Geometry: final body of the model. Coordinates: model frame, mm. Face numbers are marked on the shaded views. A direction names the side the tool comes from. Give positions to 0.01 mm unless a question says otherwise; leave off trailing zeros. Write each loop counter-clockwise with the first axis right and the second up, starting at its lowest first coordinate (ties: lowest second). Pieces come first, ordered by that corner, then holes. Notation, with made-up numbers: M 18.5,49.25 L 40.5,49.25 A34 cw 40.5,82.25 Z; hole C 52.25,89.5 d10. An arc over 180 degrees is marked long. Use one line per item in the form item = value. Start each with the question number.
Item 1: Section query A-A on y = 2.7. Return loops of the section in (x, z).
Item 2: Contact query for flat-ended pins moving along their axis: P1, Ø1.5, axis at y = 2.5, z = 1.5, coming from the -X side; P2, Ø1, axis at y = 4, z = 4, coming from the -X side. Output: stop coordinate, or through.
Item 3: Material intervals for line 1 along X through (y, z) = (2.75, 3); line 2 along Y through (x, z) = (4, 0.5); line 3 along X through (y, z) = (3.1, 2.1), sorted ascending. Write a range as from..to.
Item 4: Section query B-B on y = 1.5. Return loops of the section in (x, z).
Item 5: Section query C-C on y = 0.6. Return loops of the section in (x, z), then the cut area to 3 significant figures.
Item 6: Pull-direction query (Z, two-part tool) for the marked faces 1, 2, 3 and 4; classes: released by +Z, released by -Z, zero draft, split by the parting line, or undercut.
Item 7: Access query for the marked faces 5, 6, 7 and 8. Directions: +Z, -Z, +X, -X, +Y, -Y. A direction counts if a zero-diameter tool reaches every point of the face in a straight line with its end or side. Return the directions, or none.
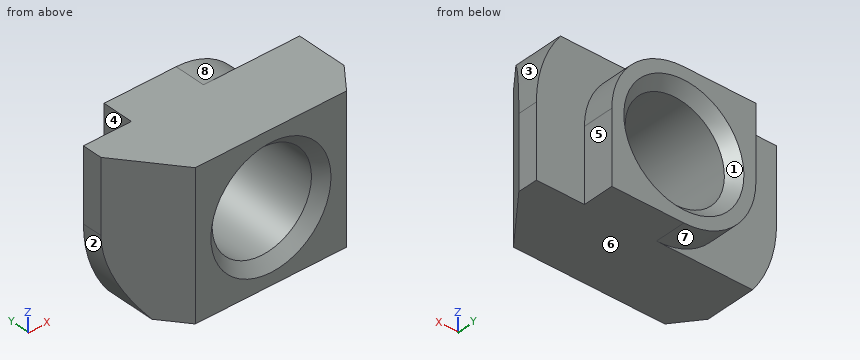
from build123d import *

# Parameters (mm, degrees)
EXTRUDE_1_DEPTH     = 6
CUT_EXTRUDE_1_DEPTH = 4.5
CUT_EXTRUDE_2_DEPTH = 4.5
FILLET_1_R          = 3


with BuildPart() as part:
    # 草图1 → 凸台-拉伸1 (new body)
    with BuildSketch(Plane.XY):
        Polygon((-5, 2.36789202), (-3.15, 0), (3.15, 0), (5, 2.36789202), (5, 3.2), (3, 3.2), (3, 4.5), (-3, 4.5), (-3, 3.2), (-5, 3.2), align=None)
    extrude(amount=EXTRUDE_1_DEPTH)

    # 草图2 → 切除-旋转1 (revolve, cut)
    with BuildSketch(Plane(origin=(0, 0, 0), x_dir=(0, 0, -1), z_dir=(1, 0, 0)), mode=Mode.PRIVATE) as cut_revolve_1_sk:
        Polygon((-3, 0), (-5.5, 0), (-5.067, 0.433), (-5.067, 4.067), (-5.5, 4.5), (-3, 4.5), align=None)
    revolve(cut_revolve_1_sk.sketch.rotate(Axis((0, 50, 3), (0, -1, 0)), 180), axis=Axis((0, 50, 3), (0, -1, 0)), mode=Mode.SUBTRACT)

    # 草图3 → 切除-拉伸1 (cut)
    with BuildSketch(Plane(origin=(0, 4.5, 0), x_dir=(1, 0, 0), z_dir=(0, 1, 0))):
        with BuildLine():
            Line((4, -6), (5, -6))
            Line((5, -6), (5, -3))
            ThreePointArc((5, -3), (4.74341649, -4.58113883), (4, -6))
        make_face()
    extrude(amount=-CUT_EXTRUDE_1_DEPTH, mode=Mode.SUBTRACT)

    # 草图4 → 切除-拉伸2 (cut)
    with BuildSketch(Plane(origin=(0, 4.5, 0), x_dir=(1, 0, 0), z_dir=(0, 1, 0))):
        with BuildLine():
            Line((-4, 0), (-5, 0))
            Line((-5, 0), (-5, -3))
            ThreePointArc((-5, -3), (-4.74341649, -1.41886117), (-4, 0))
        make_face()
    extrude(amount=-CUT_EXTRUDE_2_DEPTH, mode=Mode.SUBTRACT)

    # 圆角1
    fillet_1_edges = [part.edges().sort_by_distance(p)[0] for p in [
        (3, 3.85, 6),
        (-3, 3.85, 0),
    ]]
    fillet(fillet_1_edges, radius=FILLET_1_R)


solid = part.part
Answer sheet:
q1.outline = M -5,3 A5 ccw -4,0 L 5,0 L 5,3 A5 ccw 4,6 L -5,6 Z; hole C 0,3 d4.13
q2.P1 = -4.94
q2.P2 = -3
q3.line_1 = -5..-2.07, 2.07..5
q3.line_2 = 1.09..3.2
q3.line_3 = -4.92..-1.86, 1.86..5
q4.outline = M -4.32,0.49 A5 ccw -4,0 L 4.32,0 L 4.32,5.51 A5 ccw 4,6 L -4.32,6 Z; hole C 0,3 d4.13
q5.outline = M -3.62,0 L 3.62,0 L 3.62,6 L -3.62,6 Z; hole C 0,3 d4.13
q5.area = 30.0 mm2
q6.face_1 = undercut
q6.face_2 = released by -Z
q6.face_3 = released by +Z
q6.face_4 = zero draft
q7.face_5 = +Z, -Z, +X, +Y
q7.face_6 = -Z, +X, -X, +Y, -Y
q7.face_7 = -Z, -X, +Y
q7.face_8 = +Z, +X, +Y
